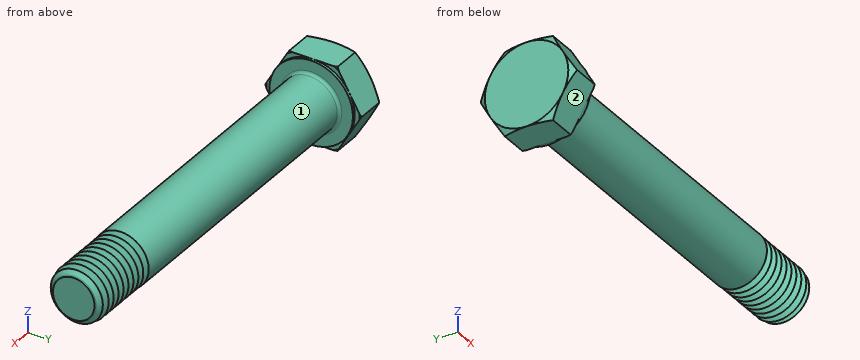
from build123d import *

# Parameters (mm, degrees)
EXTRUDE_364_DEPTH      = 7.5
SKETCH_4_W             = 0.6
SKETCH_4_H             = 11.392304845
CHAMFER_2049_SIZE      = 1.4
FILLET_2094_R          = 0.6
PATTERN_LINEAR_1_COUNT = 10
PATTERN_LINEAR_1_PITCH = 1.666666667


with BuildPart() as part:
    # 草图1 → Extrude 364 (new body)
    with BuildSketch(Plane(origin=(0, 0, 0), x_dir=(0, 0, -1), z_dir=(1, 0, 0))):
        Polygon((9, 5.196152423), (9, -5.196152423), (0, -10.392304845), (-9, -5.196152423), (-9, 5.196152423), (0, 10.392304845), align=None)
    extrude(amount=EXTRUDE_364_DEPTH)

    # 草图2 → 凸台-旋转1 (revolve)
    with BuildSketch(Plane.XY, mode=Mode.PRIVATE) as revolve_1_sk:
        Polygon((0, 0), (87.5, 0), (87.5, 4.4845), (87.5, 6), (7.791693541, 6), (0, 6), align=None)
    revolve(revolve_1_sk.sketch.rotate(Axis((0, 0, 0), (1, 0, 0)), 90), axis=Axis((0, 0, 0), (1, 0, 0)))

    # 草图3 → 切除-旋转1 (revolve, cut)
    with BuildSketch(Plane.XY):
        Polygon((0, 9), (3.690598923, 15.392304845), (3.690598923, 20.392304845), (-10, 20.392304845), (-10, 9), align=None)
    revolve(axis=Axis((0, 0, 0), (1, 0, 0)), mode=Mode.SUBTRACT)

    # 草图5 → 切除-旋转2 (revolve, cut)
    with BuildSketch(Plane.XY):
        Polygon((7.5, 9), (3.809401077, 15.392304845), (3.809401077, 20.392304845), (13.809401077, 20.392304845), (13.809401077, 9), align=None)
    revolve(axis=Axis((0, 0, 0), (1, 0, 0)), mode=Mode.SUBTRACT)

    # 草图4 → 切除-旋转3 (revolve, cut)
    with BuildSketch(Plane.XY, mode=Mode.PRIVATE) as cut_revolve_3_sk:
        with Locations((7.2, 14.696152423)):
            Rectangle(SKETCH_4_W, SKETCH_4_H)
    revolve(cut_revolve_3_sk.sketch.rotate(Axis((0, 0, 0), (1, 0, 0)), 270), axis=Axis((0, 0, 0), (1, 0, 0)), mode=Mode.SUBTRACT)

    # Chamfer 2049
    chamfer_2049_edges = [part.edges().sort_by_distance(p)[0] for p in [
        (87.5, 0, -6),
    ]]
    chamfer(chamfer_2049_edges, length=CHAMFER_2049_SIZE)

    # Fillet 2094
    fillet_2094_edges = [part.edges().sort_by_distance(p)[0] for p in [
        (7.5, 0, -6),
    ]]
    fillet(fillet_2094_edges, radius=FILLET_2094_R)

    # 草图6 → 切除-旋转4 (revolve, cut)
    with BuildSketch(Plane.XY):
        Polygon((72.5, -4.4845), (71.625025667, -6), (71.625025667, -7.5), (73.374974333, -7.5), (73.374974333, -6), align=None)
    cut_revolve_4 = revolve(axis=Axis((-3.175, 0, 0), (1, 0, 0)), mode=Mode.SUBTRACT)

    # 阵列(线性)1: 切除-旋转4 ×10
    with Locations(*[(i * PATTERN_LINEAR_1_PITCH, 0, 0) for i in range(1, PATTERN_LINEAR_1_COUNT)]):
        add(cut_revolve_4, mode=Mode.SUBTRACT)


solid = part.part
Can you work these out from the model? Positions are in its coordinate system, mm. Face numbers are marked on the shaded views. A direction names the side the tool comes from. Coordinates: 2 decimals unless noted, no trailing zeros. Loops run counter-clockwise (first coordinate to the right, second up) from the corner with the lowest first, then second, coordinate; pieces in that order, holes last. Notation, with made-up numbers: M 76,53 L 124,53 A3 ccw 124,57 Z; hole C 1,43.5 d1. An arc over 180 degrees is marked long. Return JSON: item names as keys, results as strings. Group by question number.
Item 1: On a 3-axis mill with a long thin cutter (end or side, diameter ignored), from which of +Z, -Z, +X, -X, +Y, -Y can I reach the whole of each face in a straight line? I mean the marked faces 1 and 2. Say none if no direction works.
Item 2: If I drill on L1, parallel to Y at x = 14, z = 4; L2, parallel to X at y = -5, z = -5.25; L3, parallel to Y at x = 45.5, z = 3, over which ranges is the centre line in solid material (lowest first)? Write a range as from..to.
Item 3: I'm going to push flat-ended pins straight in: pin 1 Ø1.8 at (y, z) = (-8.5, 1) entering from +X; pin 2 Ø1.3 at (y, z) = (2.5, -6) entering from +X; pin 3 Ø3.5 at (y, z) = (-2, -6.5) entering from +X. Where does each tip first touch, or does it pass through?
Item 4: Imagine slicing it at A-A (x = 52). Please give me the cut outline in (y, z).
Verdict:
{
 "1": {"face 1": "+X", "face 2": "-Z, +X, -X, -Y"},
 "2": {"L1": "y = -4.47..4.47", "L2": "x = 0..7.5", "L3": "y = -5.2..5.2"},
 "3": {"pin 1": "stops at x = 7.5", "pin 2": "stops at x = 85.04", "pin 3": "stops at x = 87.05"},
 "4": {"outline": "C 0,0 d12"}
}
